Could you check a few things on this model? Use its own coordinates, in mm. Give positions to 0.01 mm unless a question says otherwise; leave off trailing zeros. Order: outer loops, then holes, each group sorted by start corner. A loop starts at its lowest first (then second) coordinate and runs counter-clockwise, first axis right, second up. Notation, with made-up numbers: (71.5, -17) -> (96.5, -17) arc R30 cw to (96.5, 7) -> close; hole circle Ø6 at (-39.5, 59.5). An arc over 180 degrees is marked (long way). One line per item, written item: value.
```python
from build123d import *

# Parameters (mm, degrees)
EXTRUDE_1_DEPTH = 2
CHAMFER_1_SIZE  = 3


with BuildPart() as part:
    # 草图1 → 凸台-拉伸1 (new body)
    with BuildSketch(Plane.XY):
        Polygon((0, 0), (53.5, 0), (53.5, -32), (10, -60), (0, -60), align=None)
    extrude(amount=EXTRUDE_1_DEPTH)

    # 倒角1
    chamfer_1_edges = [part.edges().sort_by_distance(p)[0] for p in [
        (0, 0, 1),
        (53.5, 0, 1),
    ]]
    chamfer(chamfer_1_edges, length=CHAMFER_1_SIZE)


solid = part.part
```
1) We'd pull the mould along Y, two halves only. Please class faces 1 (the flat face through (32.054, -45.804, 0.986)), 2 (the flat face through (52, -1.5, 1)), 3 (the flat face through (27, -23, 2)): +Y half, -Y half, draft (parallel to the pull), parting line (faces both ways), or undercut.
Answer below:
face 1: -Y half
face 2: +Y half
face 3: draft
2) Suppose I cut it at A-A, the plane z = 0.3. Write out the boundary of the cut face in (x, y), then the cut area to 3 significant figures.
Answer below:
outline: (0, -60) -> (10, -60) -> (53.5, -32) -> (53.5, -3) -> (50.5, 0) -> (3, 0) -> (0, -3) -> close
area: 2,590 mm2
3) Suppose I cut it at B-B, the plane y = -46. Write out the boundary of the cut face in (x, z), then the cut area to 3 significant figures.
Answer below:
outline: (0, 0) -> (31.75, 0) -> (31.75, 2) -> (0, 2) -> close
area: 63.5 mm2
4) Suppose I cut it at C-C, the plane x = 49. Write out the boundary of the cut face in (y, z), then the cut area to 3 significant figures.
Answer below:
outline: (-34.9, 0) -> (0, 0) -> (0, 2) -> (-34.9, 2) -> close
area: 69.8 mm2
5) If I drill on line 1 along X through (y, z) = (-55, 0.9); line 2 along Y through (x, z) = (27.5, 0.5); line 3 along Y through (x, z) = (31.5, 0.35), over which ranges is the centre line in solid material (lowest first)?
Answer below:
line 1: x = 0 to 17.77
line 2: y = -48.74 to 0
line 3: y = -46.16 to 0
